Answer from the drawing. Dimensions are ordinates in mm from the lowest x, y and z of the part. A direction names the side the tool comes from. Round coordinates to 2 decimals unless told otherwise and drop trailing zeros. Write each loop counter-clockwise with the first axis right and the second up, starting at its lowest first coordinate (ties: lowest second). Pieces come first, ordered by that corner, then holes. Notation, with made-up numbers: M 77.25,-35.5 L 83.25,-35.5 A17 cw 83.25,-9.5 Z; hole C 13,28 d9. An arc over 180 degrees is marked long. One line per item, written item: value. Start each with the question number.
(1) Section A-A (x = 8) is taken. Determine the outline of the cut face in (y, z).
(2) Section D-D (x = 15) is taken. Determine the outline of the cut face in (y, z).
(3) For the marked faces 1 and 2, determine the directions among +Z, -Z, +X, -X, +Y, -Y from which every point of the face is accessible in a straight line to the end or side of a thin tool.
(4) Section C-C (y = 39) is taken. Determine the outline of the cut face in (x, z), plus the area to 3 significant figures.
(5) Consider probe 1 along Z at (x, y) = (8, 6); probe 2 along X at (y, z) = (68, 13.75); probe 3 along X at (y, z) = (12, 5.5). Determine where each line is inside the solid, lowest interval first.
(6) Given P1, Ø8, axis at y = 129, z = 8.5, coming from the -X side; P2, Ø6, axis at x = 20.5, z = 8.5, coming from the +Y side, each flat-ended and moving along its own axis, determine where each tip first touches the part or whether it passes through.
(7) Section B-B (z = 7) is taken. Determine the outline of the cut face in (x, y), plus the area to 3 significant figures.
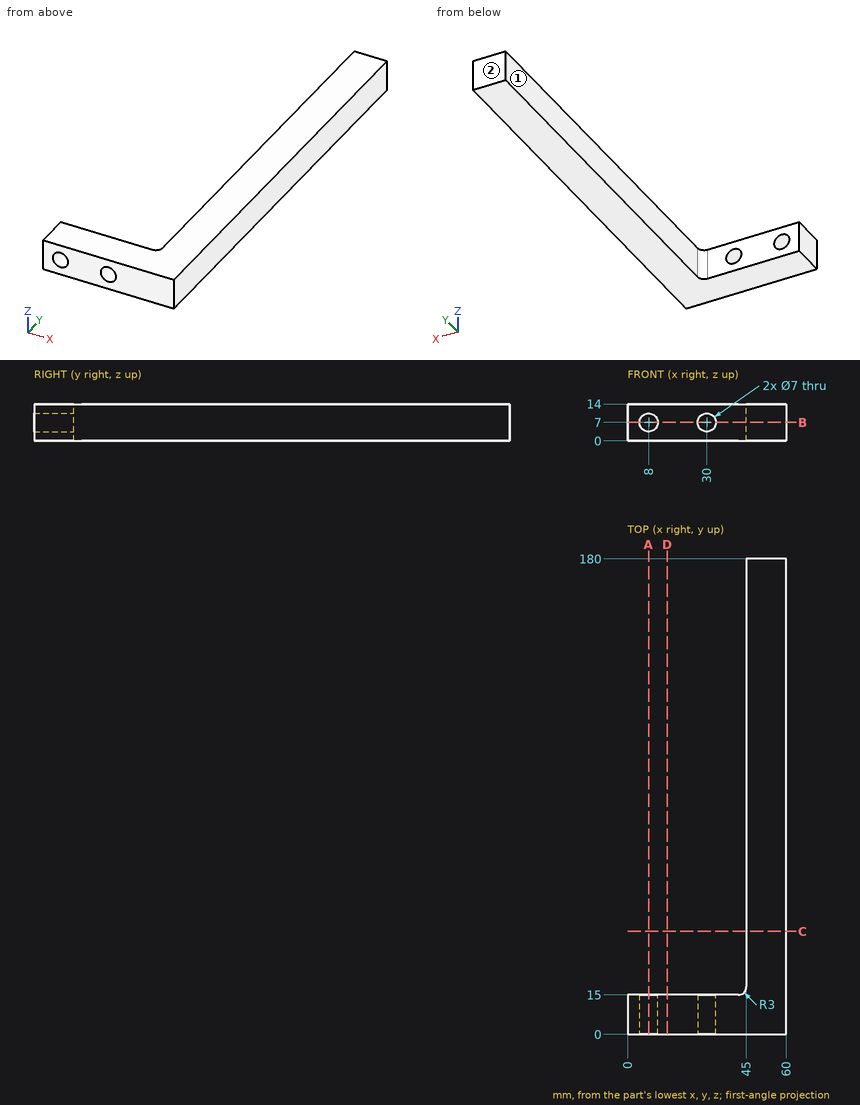
Recorded:
1. outline: M 0,0 L 15,0 L 15,3.5 L 0,3.5 Z; M 0,10.5 L 15,10.5 L 15,14 L 0,14 Z
2. outline: M 0,0 L 15,0 L 15,14 L 0,14 Z
3. face 1: +Z, -Z, -X, +Y
3. face 2: +Z, -Z, +X, -X, +Y
4. outline: M 45,0 L 60,0 L 60,14 L 45,14 Z
4. area: 210 mm2
5. probe 1: z = 0 to 3.5, 10.5 to 14
5. probe 2: x = 45 to 60
5. probe 3: x = 0 to 4.84, 11.16 to 26.84, 33.16 to 60
6. P1: stops at x = 45
6. P2: stops at y = 15
7. outline: M 0,0 L 4.5,0 L 4.5,15 L 0,15 Z; M 11.5,0 L 26.5,0 L 26.5,15 L 11.5,15 Z; M 33.5,0 L 60,0 L 60,180 L 45,180 L 45,18 A3 cw 42,15 L 33.5,15 Z
7. area: 3,170 mm2
